from build123d import *

# Parameters (mm, degrees)
SKETCH_1_R      = 2.1
SKETCH_1_R_2    = 3.4
EXTRUDE_1_DEPTH = 1000


with BuildPart() as part:
    # 草图1 → 拉伸1 (new body)
    with BuildSketch(Plane(origin=(0, 0, 0), x_dir=(1, 0, 0), z_dir=(0, 1, 0))):
        with BuildLine():
            Line((6.75, -28), (11, -28))
            Line((11, -28), (11, -30))
            Line((11, -30), (2, -30))
            ThreePointArc((2, -30), (0.585786438, -29.414213562), (0, -28))
            Line((0, -28), (0, -19))
            Line((0, -19), (2, -19))
            Line((2, -19), (2, -23.25))
            Line((2, -23.25), (5.335785999, -23.25))
            Line((5.335785999, -23.25), (9, -19.585785999))
            Line((9, -19.585785999), (9, -10.414214001))
            Line((9, -10.414214001), (5.335785999, -6.75))
            Line((5.335785999, -6.75), (2, -6.75))
            Line((2, -6.75), (2, -11))
            Line((2, -11), (0, -11))
            Line((0, -11), (0, -2))
            ThreePointArc((0, -2), (0.585786438, -0.585786438), (2, 0))
            Line((2, 0), (11, 0))
            Line((11, 0), (11, -2))
            Line((11, -2), (6.75, -2))
            Line((6.75, -2), (6.75, -5.335785999))
            Line((6.75, -5.335785999), (10.414214001, -9))
            Line((10.414214001, -9), (19.585785999, -9))
            Line((19.585785999, -9), (23.25, -5.335785999))
            Line((23.25, -5.335785999), (23.25, -2))
            Line((23.25, -2), (19, -2))
            Line((19, -2), (19, 0))
            Line((19, 0), (28, 0))
            ThreePointArc((28, 0), (29.414213562, -0.585786438), (30, -2))
            Line((30, -2), (30, -11))
            Line((30, -11), (28, -11))
            Line((28, -11), (28, -6.75))
            Line((28, -6.75), (24.664214001, -6.75))
            Line((24.664214001, -6.75), (21, -10.414214001))
            Line((21, -10.414214001), (21, -19.585785999))
            Line((21, -19.585785999), (24.664214001, -23.25))
            Line((24.664214001, -23.25), (28, -23.25))
            Line((28, -23.25), (28, -19))
            Line((28, -19), (30, -19))
            Line((30, -19), (30, -28))
            ThreePointArc((30, -28), (29.414213562, -29.414213562), (28, -30))
            Line((28, -30), (19, -30))
            Line((19, -30), (19, -28))
            Line((19, -28), (23.25, -28))
            Line((23.25, -28), (23.25, -24.664214001))
            Line((23.25, -24.664214001), (19.585785999, -21))
            Line((19.585785999, -21), (10.414214001, -21))
            Line((10.414214001, -21), (6.75, -24.664214001))
            Line((6.75, -24.664214001), (6.75, -28))
        make_face()
        with Locations(Location((3.375, -26.625, 0), (0, 0, 270))):
            Circle(SKETCH_1_R, mode=Mode.SUBTRACT)
        with Locations(Location((26.625, -26.625, 0), (0, 0, 270))):
            Circle(SKETCH_1_R, mode=Mode.SUBTRACT)
        with Locations(Location((15, -15, 0), (0, 0, 270))):
            Circle(SKETCH_1_R_2, mode=Mode.SUBTRACT)
        with Locations(Location((3.375, -3.375, 0), (0, 0, 270))):
            Circle(SKETCH_1_R, mode=Mode.SUBTRACT)
        with Locations(Location((26.625, -3.375, 0), (0, 0, 270))):
            Circle(SKETCH_1_R, mode=Mode.SUBTRACT)
    extrude(amount=EXTRUDE_1_DEPTH)


solid = part.part
The model under review builds one solid part; all positions refer to its coordinate system, in mm. Give positions to 0.01 mm unless a question says otherwise; leave off trailing zeros. One line per question, with ' | ' between items. Start each with the question number.
1) Wall thickness on L1, parallel to Z at x = 2.5, y = 476; L2, parallel to Z at x = 14.25, y = 208.5: over which ranges is each line inside the solid? List them lowest first. Write a range as from..to.
2) Consider section A-A, the plane y = 562. State how many separate pieces and enclosed holes the cut face has, then the cut area to 3 significant figures.
3) Clearance check with flat-ended pins moving along their axes: P1, Ø1, axis at x = 3, y = 640.5, coming from the -Z side; P2, Ø3, axis at x = 16.5, y = 340.5, coming from the -Z side; P3, Ø4, axis at y = 106, z = 15.5, coming from the +X side; P4, Ø2, axis at y = 453.5, z = 29.5, coming from the +X side. State where each tip first meets the part, or that it passes through.
Found:
1) L1: z = 0..1.47, 5.28..6.75, 23.25..24.72, 28.53..30 | L2: z = 9..11.68, 18.32..21
2) separate pieces: 1 | enclosed holes: 5 | area: 333 mm²
3) P1: stops at z = 0 | P2: stops at z = 9 | P3: stops at x = 21 | P4: stops at x = 29.94
